```python
from build123d import *

# Parameters (mm, degrees)
SKETCH_1_W          = 160
SKETCH_1_H          = 30
EXTRUDE_1_DEPTH     = 10
CHAMFER_1_SIZE      = 2
CHAMFER_2_SIZE      = 1
HOLE_WIZARD_M6_1_D  = 6.6
CUT_EXTRUDE_1_DEPTH = 83.006097334


with BuildPart() as part:
    # 草图1 → 凸台-拉伸1 (new body)
    with BuildSketch(Plane.XY):
        Rectangle(SKETCH_1_W, SKETCH_1_H)
    extrude(amount=EXTRUDE_1_DEPTH)

    # 倒角1
    chamfer_1_edges = [part.edges().sort_by_distance(p)[0] for p in [
        (-80, 15, 5),
        (80, 15, 5),
    ]]
    chamfer(chamfer_1_edges, length=CHAMFER_1_SIZE)

    # 倒角2
    chamfer_2_edges = [part.edges().sort_by_distance(p)[0] for p in [
        (80, -15, 5),
        (-80, -15, 5),
    ]]
    chamfer(chamfer_2_edges, length=CHAMFER_2_SIZE)

    # M6 间隙孔1 (through all)
    with Locations(Plane.XY.offset(10)):
        with Locations((-70, 0)):
            Hole(HOLE_WIZARD_M6_1_D / 2)

    # 草图4 → 切除-拉伸1 (cut, through all)
    with BuildSketch(Plane.XY.offset(10)):
        with BuildLine():
            Line((-7.46846906, 15), (78, 15))
            ThreePointArc((78, 15), (35.26576547, 1.017096174), (-7.46846906, 15))
        make_face()
    extrude(amount=-CUT_EXTRUDE_1_DEPTH, mode=Mode.SUBTRACT)


solid = part.part
```
Here's how the part is built. I have some questions about the finished solid (model axes, mm). Round coordinates to 2 decimals unless told otherwise and drop trailing zeros. Loops run counter-clockwise (first coordinate to the right, second up) from the corner with the lowest first, then second, coordinate; pieces in that order, holes last. Notation, with made-up numbers: (25.25, 0) -> (52.25, 0) arc R12 cw to (52.25, 23) -> close; hole circle Ø8 at (-15.5, -29.5). An arc over 180 degrees is marked (long way). Answer as CSV lines item,"result".
1. If we section it at B-B on z = 8: Please give me the cut outline in (x, y).
Final values:
outline,"(-80, -14) -> (-79, -15) -> (79, -15) -> (80, -14) -> (80, 13) -> (78, 15) arc R72.29 cw to (-7.47, 15) -> (-78, 15) -> (-80, 13) -> close; hole circle Ø6.6 at (-70, 0)"
2. If we section it at D-D on x = 0: Please give me the cut outline in (y, z).
Final values:
outline,"(-15, 0) -> (10.2, 0) -> (10.2, 10) -> (-15, 10) -> close"
3. If we section it at A-A on x = -70: Please give me the cut outline in (y, z).
Final values:
outline,"(-15, 0) -> (-3.3, 0) -> (-3.3, 10) -> (-15, 10) -> close; (3.3, 0) -> (15, 0) -> (15, 10) -> (3.3, 10) -> close"
4. Thinking about a two-plate mould opening in X: for faces 1 (the face through (-1, -3, 0)), 2 (the face through (-66.7, 0.1, 4.9)), 3 (the face through (35.91, 1.02, 5.07)), 4 (the face through (-80, -1, 5)), which applies, released by +X, released by -X, zero draft, split by the parting line, or undercut?
Final values:
face 1,"zero draft"
face 2,"undercut"
face 3,"undercut"
face 4,"released by -X"
5. For pin 1 (5 mm diameter, centred on x = 53, z = 5, fed in from +Y), with a flat end and sliding along its axis, tell me the tip position at first contact or that it passes through.
Final values:
pin 1,"stops at y = 3.91"
6. If we section it at C-C on y = 11.5: Please give me the cut outline in (x, z), plus the area to 3 significant figures.
Final values:
outline,"(-80, 0) -> (-2.23, 0) -> (-2.23, 10) -> (-80, 10) -> close; (72.76, 0) -> (80, 0) -> (80, 10) -> (72.76, 10) -> close"
area,"850 mm^2"
7. If I drill on L1, parallel to Y at x = -70, z = 6.75; L2, parallel to X at y = 7, z = 3; L3, parallel to Y at x = -68, z = 2.5, over which ranges is the centre line in solid material (lowest first)?
Final values:
L1,"y = -15 to -3.3, 3.3 to 15"
L2,"x = -80 to 6.47, 64.06 to 80"
L3,"y = -15 to -2.62, 2.62 to 15"
